Build history of the part. All positions in model axes, mm. A direction names the side the tool comes from. Coordinates: 2 decimals unless noted, no trailing zeros. Loops run counter-clockwise (first coordinate to the right, second up) from the corner with the lowest first, then second, coordinate; pieces in that order, holes last. Notation, with made-up numbers: (57, -34.75) -> (102, -34.75) arc R17 ccw to (102, -18.75) -> close; hole circle Ø5 at (-13.75, 25). An arc over 180 degrees is marked (long way). One line per item, written item: value. Start each with the question number.
```python
from build123d import *

# Parameters (mm, degrees)
SUPPORT_BODY_50MM_DEPTH    = 50
TOP_SLOT_34MM_DEEP_DEPTH   = 34
CLEVIS_NOTCH_SKETCH_W      = 30
CLEVIS_NOTCH_SKETCH_H      = 26
CLEVIS_NOTCH_DEPTH         = 117.062863291
SIDE_RELIEF_SKETCH_W       = 26
SIDE_RELIEF_SKETCH_H       = 10
SIDE_RELIEF_CUT_10MM_DEPTH = 10


with BuildPart() as part:
    # Support Profile Sketch → Support Body 50mm (new body)
    with BuildSketch(Plane.XY):
        Polygon((0, 0), (45, 0), (45, 20), (80, 20), (80, 0), (90, 0), (90, 50), (50, 50), (50, 40), (35, 40), (0, 10), align=None)
    extrude(amount=SUPPORT_BODY_50MM_DEPTH)

    # Top Slot Sketch → Top Slot 34mm Deep (cut)
    with BuildSketch(Plane(origin=(0, 50, 0), x_dir=(1, 0, 0), z_dir=(0, 1, 0))):
        with BuildLine():
            Line((76.808802697, -10.147055453), (76.808802697, -39.852944547))
            ThreePointArc((76.808802697, -39.852944547), (71.661747244, -45), (66.514691792, -39.852944547))
            Line((66.514691792, -39.852944547), (66.514691792, -10.147055453))
            ThreePointArc((66.514691792, -10.147055453), (71.661747244, -5), (76.808802697, -10.147055453))
        make_face()
    extrude(amount=-TOP_SLOT_34MM_DEEP_DEPTH, mode=Mode.SUBTRACT)

    # Clevis Notch Sketch → Clevis Notch (cut, through all)
    with BuildSketch(Plane(origin=(-4.941176471, 5.764705882, 0), x_dir=(0.7592566023652966, 0.6507913734559686, 0), z_dir=(-0.6507913734559686, 0.7592566023652966, 0))):
        with Locations((21.507913735, -25)):
            Rectangle(CLEVIS_NOTCH_SKETCH_W, CLEVIS_NOTCH_SKETCH_H)
    extrude(amount=-CLEVIS_NOTCH_DEPTH, mode=Mode.SUBTRACT)

    # Side Relief Sketch → Side Relief Cut 10mm (cut)
    with BuildSketch(Plane.ZY):
        with Locations((25, 5)):
            Rectangle(SIDE_RELIEF_SKETCH_W, SIDE_RELIEF_SKETCH_H)
    extrude(amount=-SIDE_RELIEF_CUT_10MM_DEPTH, mode=Mode.SUBTRACT)


solid = part.part
```
Item 1: Band-saw the part on B-B, the plane y = 37. List the corners of the cut face in (x, z).
Item 2: Band-saw the part on A-A, the plane z = 21.5. List the corners of the cut face in (x, y), and give its area (3 significant figures).
Item 3: Two-plate mould, pull along Z, no slides. Class faces 1 (the face through (71.55, 35.21, 5)), 2 (the face through (43, 40, 25)), 3 (the face through (54, 25, 50)): +Z half, -Z half, draft (parallel to the pull), parting line (faces both ways), or undercut.
Item 4: Tool access for faces 4 (the face through (0, 5, 6)), 5 (the face through (71.8, 35.2, 45)), 6 (the face through (21, 9, 12)), 7 (the face through (50, 45, 25)), 8 (the face through (45, 10, 25)): list every direction of +Z, -Z, +X, -X, +Y, -Y with a clear straight run to the whole face (end or side of a thin tool).
Item 5: Probe probe 1 along Z at (x, y) = (13, 11); probe 2 along X at (y, z) = (4.5, 7); probe 3 along Y at (x, z) = (51.5, 8.5). List the from-to ranges inside material, lowest first.
Item 6: Band-saw the part on C-C, the plane x = 14. List the corners of the cut face in (y, z), and give its area (3 significant figures).
Item 7: Band-saw the part on D-D, the plane z = 46. List the corners of the cut face in (x, y), and give its area (4 significant figures).
Item 8: Drop flat-ended pins along their axis: pin 1 Ø8 at (x, z) = (26, 8) entering from +Y; pin 2 Ø17.5 at (x, z) = (67, 35.5) entering from -Y; pin 3 Ø4.5 at (x, z) = (39.5, 14.5) entering from +Y. Give the stop position or say it passes through.
Worked out:
1. outline: (31.5, 0) -> (90, 0) -> (90, 50) -> (31.5, 50) -> close; hole (66.51, 10.15) arc R5.15 ccw to (76.81, 10.15) -> (76.81, 39.85) arc R5.15 ccw to (66.51, 39.85) -> close
2. outline: (22.78, 29.52) -> (45, 3.6) -> (45, 20) -> (66.51, 20) -> (66.51, 50) -> (50, 50) -> (50, 40) -> (35, 40) -> close; (76.81, 20) -> (80, 20) -> (80, 0) -> (90, 0) -> (90, 50) -> (76.81, 50) -> close
2. area: 1,650 mm²
3. face 1: undercut
3. face 2: draft
3. face 3: +Z half
4. face 4: +Z, -Z, -X, +Y, -Y
4. face 5: +Y, -Y
4. face 6: -X, -Y
4. face 7: +Z, -Z, -X, +Y
4. face 8: +Z, -Z, -Y
5. probe 1: z = 0 to 12, 38 to 50
5. probe 2: x = 0 to 45, 80 to 90
5. probe 3: y = 20 to 50
6. outline: (0, 0) -> (22, 0) -> (22, 12) -> (0, 12) -> close; (0, 38) -> (22, 38) -> (22, 50) -> (0, 50) -> close
6. area: 528 mm²
7. outline: (0, 0) -> (45, 0) -> (45, 20) -> (80, 20) -> (80, 0) -> (90, 0) -> (90, 50) -> (50, 50) -> (50, 40) -> (35, 40) -> (0, 10) -> close
7. area: 2,775 mm²
8. pin 1: stops at y = 35.71
8. pin 2: stops at y = 20
8. pin 3: stops at y = 40
